```python
from build123d import *

# Parameters (mm, degrees)
BASE_PLATE_SKETCH_W                       = 200
BASE_PLATE_SKETCH_H                       = 213
BASE_PLATE_DEPTH                          = 25
BOLT_PAD_DEPTH                            = 10
BASE_PLATE_FILLETS_R10_R                  = 10
CENTRAL_HOUSING_DEPTH                     = 95
BEARING_BOSS_A_DEPTH                      = 10
BEARING_BOSS_A_DEPTH_BACK                 = 120
BEARING_BOSS_A_SKETCH_R                   = 35
BEARING_BOSS_B_DEPTH                      = 10
BEARING_BOSS_B_DEPTH_BACK                 = 120
BEARING_BOSS_B_SKETCH_R                   = 41.5
BEARING_BORE_A_41_REACH                   = 298.498
BEARING_BORE_A_SKETCH_R                   = 20.5
BEARING_BORE_B_41_REACH                   = 291.404
BEARING_BORE_B_SKETCH_R                   = 20.5
BORE_CHAMFERS_2X45_SIZE                   = 2
M8_COUNTERBORED_MOUNTING_HOLE_D           = 15
M8_COUNTERBORED_MOUNTING_HOLE_CBORE_D     = 30
M8_COUNTERBORED_MOUNTING_HOLE_CBORE_DEPTH = 10
BASE_POCKET_DEPTH                         = 20


with BuildPart() as part:
    # Base Plate Sketch → Base Plate (new body)
    with BuildSketch(Plane(origin=(0, 0, 0), x_dir=(1, 0, 0), z_dir=(0, 1, 0))):
        Rectangle(BASE_PLATE_SKETCH_W, BASE_PLATE_SKETCH_H)
    extrude(amount=BASE_PLATE_DEPTH)

    # Bolt Pad Sketch → Bolt Pad (add)
    with BuildSketch(Plane(origin=(0, 25, 0), x_dir=(1, 0, 0), z_dir=(0, 1, 0))):
        with BuildLine():
            Line((100, -106.5), (40, -106.5))
            Line((40, -106.5), (40, -61.5))
            ThreePointArc((40, -61.5), (44.393398282, -50.893398282), (55, -46.5))
            Line((55, -46.5), (100, -46.5))
            Line((100, -46.5), (100, -106.5))
        make_face()
    extrude(amount=BOLT_PAD_DEPTH)

    # Base Plate Fillets R10
    base_plate_fillets_r10_edges = [part.edges().sort_by_distance(p)[0] for p in [
        (100, 17.5, 106.5),
        (-100, 12.5, 106.5),
        (-100, 12.5, -106.5),
        (100, 12.5, -106.5),
    ]]
    fillet(base_plate_fillets_r10_edges, radius=BASE_PLATE_FILLETS_R10_R)

    # Central Housing Sketch → Central Housing (add)
    with BuildSketch(Plane(origin=(0, 25, 0), x_dir=(1, 0, 0), z_dir=(0, 1, 0))):
        with BuildLine():
            Line((100, 63.5), (20, 63.5))
            ThreePointArc((20, 63.5), (-6.360389693, -0.139610307), (-70, -26.5))
            Line((-70, -26.5), (-70, -106.5))
            Line((-70, -106.5), (-55, -106.5))
            Line((-55, -106.5), (-55, -40.423048454))
            ThreePointArc((-55, -40.423048454), (4.246212025, -10.746212025), (33.923048454, 48.5))
            Line((33.923048454, 48.5), (100, 48.5))
            Line((100, 48.5), (100, 63.5))
        make_face()
    extrude(amount=CENTRAL_HOUSING_DEPTH)

    # Bearing Boss A Sketch → Bearing Boss A (add, two sides: drawn at the far end of the back side and taken through both)
    with BuildSketch(Plane.XY.offset(106.5).offset(-BEARING_BOSS_A_DEPTH_BACK)):
        with Locations((-62.5, 120)):
            Circle(BEARING_BOSS_A_SKETCH_R)
    extrude(amount=BEARING_BOSS_A_DEPTH + BEARING_BOSS_A_DEPTH_BACK)

    # Bearing Boss B Sketch → Bearing Boss B (add, two sides: drawn at the far end of the back side and taken through both)
    with BuildSketch(Plane(origin=(100, 0, 0), x_dir=(0, 0, -1), z_dir=(1, 0, 0)).offset(-BEARING_BOSS_B_DEPTH_BACK)):
        with Locations((56, 120)):
            Circle(BEARING_BOSS_B_SKETCH_R)
    extrude(amount=BEARING_BOSS_B_DEPTH + BEARING_BOSS_B_DEPTH_BACK)

    # Bearing Bore A Sketch → Bearing Bore A Ø41 (cut, up to next)
    with BuildSketch(Plane.XY.offset(116.5), mode=Mode.PRIVATE) as bearing_bore_a_41_sk1:
        with Locations((-62.5, 120)):
            Circle(BEARING_BORE_A_SKETCH_R)
    bearing_bore_a_41_tool1 = extrude(bearing_bore_a_41_sk1.sketch, amount=-BEARING_BORE_A_41_REACH, mode=Mode.PRIVATE) & part.part
    add(bearing_bore_a_41_tool1.solids().sort_by_distance((-62.5, 120, 116.5))[0], mode=Mode.SUBTRACT)

    # Bearing Bore B Sketch → Bearing Bore B Ø41 (cut, up to next)
    with BuildSketch(Plane(origin=(110, 0, 0), x_dir=(0, 0, -1), z_dir=(1, 0, 0)), mode=Mode.PRIVATE) as bearing_bore_b_41_sk1:
        with Locations((56, 120)):
            Circle(BEARING_BORE_B_SKETCH_R)
    bearing_bore_b_41_tool1 = extrude(bearing_bore_b_41_sk1.sketch, amount=-BEARING_BORE_B_41_REACH, mode=Mode.PRIVATE) & part.part
    add(bearing_bore_b_41_tool1.solids().sort_by_distance((110, 120, -56))[0], mode=Mode.SUBTRACT)

    # Bore Chamfers 2x45°
    bore_chamfers_2x45_edges = [part.edges().sort_by_distance(p)[0] for p in [
        (-83, 120, 116.5),
        (-83, 120, -13.5),
        (110, 120, -35.5),
        (-20, 120, -35.5),
    ]]
    chamfer(bore_chamfers_2x45_edges, length=BORE_CHAMFERS_2X45_SIZE)

    # M8 Counterbored Mounting Hole (through all)
    with Locations(Plane(origin=(70, 35, 76.5), x_dir=(0, 0, 1), z_dir=(0, 1, 0))):
        with Locations((0, 0)):
            CounterBoreHole(M8_COUNTERBORED_MOUNTING_HOLE_D / 2, M8_COUNTERBORED_MOUNTING_HOLE_CBORE_D / 2, M8_COUNTERBORED_MOUNTING_HOLE_CBORE_DEPTH)

    # Base Pocket Sketch → Base Pocket (cut)
    with BuildSketch(Plane(origin=(0, 25, 0), x_dir=(1, 0, 0), z_dir=(0, 1, 0))):
        with BuildLine():
            Line((-46, -55.747641486), (-46, -87.5))
            ThreePointArc((-46, -87.5), (-43.071067812, -94.571067812), (-36, -97.5))
            Line((-36, -97.5), (21, -97.5))
            ThreePointArc((21, -97.5), (28.071067812, -94.571067812), (31, -87.5))
            Line((31, -87.5), (31, -61.5))
            ThreePointArc((31, -61.5), (38.029437252, -44.529437252), (55, -37.5))
            Line((55, -37.5), (81, -37.5))
            ThreePointArc((81, -37.5), (88.071067812, -34.571067812), (91, -27.5))
            Line((91, -27.5), (91, 29.5))
            ThreePointArc((91, 29.5), (88.071067812, 36.571067812), (81, 39.5))
            Line((81, 39.5), (49.247641486, 39.5))
            ThreePointArc((49.247641486, 39.5), (43.223496519, 37.481834214), (39.630896205, 32.241935484))
            ThreePointArc((39.630896205, 32.241935484), (10.610173055, -17.110173055), (-38.741935484, -46.130896205))
            ThreePointArc((-38.741935484, -46.130896205), (-43.981834214, -49.723496519), (-46, -55.747641486))
        make_face()
    extrude(amount=-BASE_POCKET_DEPTH, mode=Mode.SUBTRACT)


solid = part.part
```
Check sheet for the modelled part. Datum: model origin and axes. Units: mm. A direction names the side the tool comes from. Give positions to 0.01 mm unless a question says otherwise; leave off trailing zeros. Loops run counter-clockwise (first coordinate to the right, second up) from the corner with the lowest first, then second, coordinate; pieces in that order, holes last. Notation, with made-up numbers: M -14.5,58 L 2.5,58 A20 ccw 2.5,64 Z; hole C 19,50.25 d7. An arc over 180 degrees is marked long. Answer in a Markdown table with one row per item.
1) Depth check by flat-ended pin: pin 1 (10 mm diameter, centred on x = 44, y = 83.5, fed in from -Z); pin 2 (18 mm diameter, centred on x = 70, z = 76.5, fed in from +Y); pin 3 (5 mm diameter, centred on x = 79, y = 128, fed in from -Z); pin 4 (9 mm diameter, centred on x = 70, z = 76.5, fed in from -Y). Enter the tip coordinate at first touch or a pass-through.
Solutions:
| item | result |
|---|---|
| pin 1 | stops at z = -83.02 |
| pin 2 | stops at y = 25 |
| pin 3 | stops at z = -97.13 |
| pin 4 | passes through |
2) Mould release check, pull along Y, two halves, no side actions. Record for faces 4 (the face through (3.576, 61.279, 11.411)), 5 (the face through (-96.99, 12.68, -103.65)), 6 (the face through (-1, 0, -1)): released by +Y, released by -Y, zero draft, split by the parting line, or undercut.
Solutions:
| item | result |
|---|---|
| face 4 | undercut |
| face 5 | zero draft |
| face 6 | released by -Y |
3) Cross-section at A-A (x = 70). Enter the section's corners in (y, z).
Solutions:
| item | result |
|---|---|
| outline | M 0,-106.5 L 25,-106.5 L 25,-63.5 L 79.18,-63.5 A41.5 ccw long 79.18,-48.5 L 25,-48.5 L 25,-39.5 L 5,-39.5 L 5,37.5 L 25,37.5 L 25,46.5 L 35,46.5 L 35,61.5 L 25,61.5 L 25,69 L 0,69 Z; M 0,84 L 25,84 L 25,91.5 L 35,91.5 L 35,106.5 L 0,106.5 Z; hole C 120,-56 d41 |
4) Tool access check on faces 1 (the face through (-96.99, 12.68, 103.65)), 2 (the face through (-3, 120, 9)), 3 (the face through (43.3, 15.14, -37.54)). Record the directions out of +Z, -Z, +X, -X, +Y, -Y that give a thin tool (end or side, any length) a straight path to the whole face; none if there is none.
Solutions:
| item | result |
|---|---|
| face 1 | +Z, -X, -Y |
| face 2 | +Z, +X, +Y |
| face 3 | none |
5) Cross-section at D-D (z = -56). Enter the section's corners in (x, y), plus the area to 3 significant figures.
Solutions:
| item | result |
|---|---|
| outline | M -100,0 L 100,0 L 100,78.5 L 110,78.5 L 110,97.5 L 108,99.5 L -18,99.5 L -20,97.5 L -20,78.5 L 19.69,78.5 L 19.69,25 L -100,25 Z; M -20,142.5 L -18,140.5 L 108,140.5 L 110,142.5 L 110,161.5 L -20,161.5 Z |
| area | 14,700 mm^2 |
6) Thickness scan on line 1 (X direction, y = 27, z = 76); line 2 (Y direction, x = -62.5, z = 17.5); line 3 (X direction, y = 13.25, z = 76.5). Record the ranges inside material, lowest first.
Solutions:
| item | result |
|---|---|
| line 1 | x = -70 to -55, 40 to 55.01, 84.99 to 100 |
| line 2 | y = 0 to 25, 85 to 99.5, 140.5 to 155 |
| line 3 | x = -100 to -46, 31 to 62.5, 77.5 to 100 |
7) Cross-section at B-B (z = 76.5). Enter the section's corners in (x, y), plus the area to 3 significant figures.
Solutions:
| item | result |
|---|---|
| outline | M -100,0 L 62.5,0 L 62.5,25 L 55,25 L 55,35 L 40,35 L 40,25 L 31,25 L 31,5 L -46,5 L -46,25 L -55,25 L -55,85.81 A35 ccw long -70,85.81 L -70,25 L -100,25 Z; M 77.5,0 L 100,0 L 100,35 L 85,35 L 85,25 L 77.5,25 Z; hole C -62.5,120 d41 |
| area | 6,820 mm^2 |
8) Cross-section at C-C (y = 43). Enter the section's corners in (x, z), plus the area to 3 significant figures.
Solutions:
| item | result |
|---|---|
| outline | M -70,26.5 A90 cw 20,-63.5 L 100,-63.5 L 100,-48.5 L 33.92,-48.5 A105 ccw -55,40.42 L -55,106.5 L -70,106.5 Z |
| area | 4,260 mm^2 |
